```python
from build123d import *

# Parameters (mm, degrees)
SKETCH3_R           = 25
SKETCH3_R_2         = 72
BOSS_EXTRUDE1_DEPTH = 28
SKETCH4_R           = 10.5
CUT_EXTRUDE1_DEPTH  = 3671.216984417


with BuildPart() as part:
    # Sketch3 → Boss-Extrude1 (new body)
    with BuildSketch(Plane(origin=(0, 0, 0), x_dir=(1, 0, 0), z_dir=(0, 1, 0))):
        with BuildLine():
            Line((2845.680118699, 2169.501165066), (2845.680118699, 2074.501165066))
            ThreePointArc((2845.680118699, 2074.501165066), (2848.414414178, 2016.917733414), (2860.484776028, 1960.547223948))
            ThreePointArc((2860.484776028, 1960.547223948), (2949.180118699, 1699.501165066), (2860.484776028, 1438.455106185))
            ThreePointArc((2860.484776028, 1438.455106185), (2848.414414178, 1382.084596719), (2845.680118699, 1324.501165066))
            Line((2845.680118699, 1324.501165066), (2845.680118699, 1229.501165066))
            Line((2845.680118699, 1229.501165066), (2830.680118699, 1214.501165066))
            Line((2830.680118699, 1214.501165066), (2210.680118699, 1214.501165066))
            Line((2210.680118699, 1214.501165066), (2195.680118699, 1229.501165066))
            Line((2195.680118699, 1229.501165066), (2195.680118699, 1324.501165066))
            ThreePointArc((2195.680118699, 1324.501165066), (2192.94582322, 1382.084596719), (2180.87546137, 1438.455106185))
            ThreePointArc((2180.87546137, 1438.455106185), (2092.180118699, 1699.501165066), (2180.87546137, 1960.547223948))
            ThreePointArc((2180.87546137, 1960.547223948), (2192.94582322, 2016.917733414), (2195.680118699, 2074.501165066))
            Line((2195.680118699, 2074.501165066), (2195.680118699, 2169.501165066))
            Line((2195.680118699, 2169.501165066), (2210.680118699, 2184.501165066))
            Line((2210.680118699, 2184.501165066), (2830.680118699, 2184.501165066))
            Line((2830.680118699, 2184.501165066), (2845.680118699, 2169.501165066))
        make_face()
        with Locations(Location((2844.180118699, 1699.501165066, 0), (0, 0, 270))):
            Circle(SKETCH3_R, mode=Mode.SUBTRACT)
        with Locations(Location((2520.680118699, 1400.501165066, 0), (0, 0, 270))):
            Circle(SKETCH3_R_2, mode=Mode.SUBTRACT)
        with Locations(Location((2520.680118699, 1998.501165066, 0), (0, 0, 270))):
            Circle(SKETCH3_R_2, mode=Mode.SUBTRACT)
        with BuildLine():
            Line((2620.554891012, 1673.06787727), (2562.676931085, 1635.306037562))
            ThreePointArc((2562.676931085, 1635.306037562), (2520.680118699, 1622.914580714), (2478.683306313, 1635.306037562))
            Line((2478.683306313, 1635.306037562), (2420.805346386, 1673.06787727))
            ThreePointArc((2420.805346386, 1673.06787727), (2406.139786968, 1699.889370895), (2420.805346386, 1726.71086452))
            Line((2420.805346386, 1726.71086452), (2478.683306313, 1764.472704228))
            ThreePointArc((2478.683306313, 1764.472704228), (2520.680118699, 1776.864161076), (2562.676931085, 1764.472704228))
            Line((2562.676931085, 1764.472704228), (2620.554891012, 1726.71086452))
            ThreePointArc((2620.554891012, 1726.71086452), (2635.220450429, 1699.889370895), (2620.554891012, 1673.06787727))
        make_face(mode=Mode.SUBTRACT)
    extrude(amount=BOSS_EXTRUDE1_DEPTH)

    # Sketch4 → Cut-Extrude1 (cut, through all)
    with BuildSketch(Plane(origin=(0, 28, 0), x_dir=(1, 0, 0), z_dir=(0, 1, 0))):
        with Locations(Location((2520.680118699, 2099.501165066, 0), (0, 0, 270))):
            Circle(SKETCH4_R)
        with Locations(Location((2624.20773674, 2085.871495582, 0), (0, 0, 270))):
            Circle(SKETCH4_R)
        with Locations(Location((2720.680118699, 2045.91132658, 0), (0, 0, 270))):
            Circle(SKETCH4_R)
        with Locations(Location((2803.522831173, 1982.343877541, 0), (0, 0, 270))):
            Circle(SKETCH4_R)
        with Locations(Location((2867.090280213, 1899.501165066, 0), (0, 0, 270))):
            Circle(SKETCH4_R)
        with Locations(Location((2907.050449214, 1803.028783107, 0), (0, 0, 270))):
            Circle(SKETCH4_R)
        with Locations(Location((2920.680118699, 1699.501165066, 0), (0, 0, 270))):
            Circle(SKETCH4_R)
        with Locations(Location((2907.050449214, 1595.973547025, 0), (0, 0, 270))):
            Circle(SKETCH4_R)
        with Locations(Location((2867.090280213, 1499.501165066, 0), (0, 0, 270))):
            Circle(SKETCH4_R)
        with Locations(Location((2803.522831173, 1416.658452592, 0), (0, 0, 270))):
            Circle(SKETCH4_R)
        with Locations(Location((2720.680118699, 1353.091003552, 0), (0, 0, 270))):
            Circle(SKETCH4_R)
        with Locations(Location((2624.20773674, 1313.130834551, 0), (0, 0, 270))):
            Circle(SKETCH4_R)
        with Locations(Location((2520.680118699, 1299.501165066, 0), (0, 0, 270))):
            Circle(SKETCH4_R)
        with Locations(Location((2417.152500658, 1313.130834551, 0), (0, 0, 270))):
            Circle(SKETCH4_R)
        with Locations(Location((2320.680118699, 1353.091003552, 0), (0, 0, 270))):
            Circle(SKETCH4_R)
        with Locations(Location((2237.837406224, 1416.658452592, 0), (0, 0, 270))):
            Circle(SKETCH4_R)
        with Locations(Location((2174.269957185, 1499.501165066, 0), (0, 0, 270))):
            Circle(SKETCH4_R)
        with Locations(Location((2134.309788183, 1595.973547025, 0), (0, 0, 270))):
            Circle(SKETCH4_R)
        with Locations(Location((2120.680118699, 1699.501165066, 0), (0, 0, 270))):
            Circle(SKETCH4_R)
        with Locations(Location((2134.309788183, 1803.028783107, 0), (0, 0, 270))):
            Circle(SKETCH4_R)
        with Locations(Location((2174.269957185, 1899.501165066, 0), (0, 0, 270))):
            Circle(SKETCH4_R)
        with Locations(Location((2237.837406224, 1982.343877541, 0), (0, 0, 270))):
            Circle(SKETCH4_R)
        with Locations(Location((2320.680118699, 2045.91132658, 0), (0, 0, 270))):
            Circle(SKETCH4_R)
        with Locations(Location((2417.152500658, 2085.871495582, 0), (0, 0, 270))):
            Circle(SKETCH4_R)
    extrude(amount=-CUT_EXTRUDE1_DEPTH, mode=Mode.SUBTRACT)


solid = part.part
```
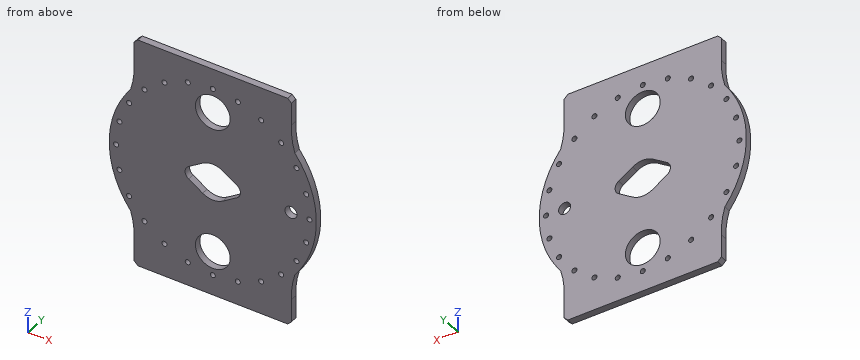
Geometry: final body of the model. Coordinates: model frame, mm. Coordinates: 2 decimals unless noted, no trailing zeros. Order: outer loops, then holes, each group sorted by start corner. A loop starts at its lowest first (then second) coordinate and runs counter-clockwise, first axis right, second up. Notation, with made-up numbers: M 60,14.25 L 87,14.25 A21 ccw 87,25.25 Z; hole C 68.5,55 d1. An arc over 180 degrees is marked long. Answer in a Markdown table with one row per item. Add a question column.
Q1. Section query A-A on z = -1596. Return the cut outline in (x, y), and give its area (3 significant figures).
Q2. Contact query for flat-ended pins moving along their axis: P1, Ø8, axis at y = 7.5, z = -2037, coming from the -X side; P2, Ø14, axis at y = 15.5, z = -1258, coming from the +X side; P3, Ø1, axis at y = 7, z = -1872, coming from the +X side. Output: stop coordinate, or through.
Q3. Section query B-B on y = 5. Count the separate pieces of the cut face and the enclosed holes in it, and give its area (3 significant figures).
Q4. Line query: L1, parallel to X at y = 27, z = -1989; L2, parallel to X at y = 14.5, z = -1422; L3, parallel to X at y = 23.25, z = -1490. Output: solid intervals per line, ascending.
Completed:
| question | item | result |
|---|---|---|
| 1 | outline | M 2104.87,0 L 2123.81,0 L 2123.81,28 L 2104.87,28 Z; M 2144.81,0 L 2896.55,0 L 2896.55,28 L 2144.81,28 Z; M 2917.55,0 L 2936.49,0 L 2936.49,28 L 2917.55,28 Z |
| 1 | area | 22,100 mm2 |
| 2 | P1 | stops at x = 2194.66 |
| 2 | P2 | stops at x = 2845.68 |
| 2 | P3 | stops at x = 2913.14 |
| 3 | separate pieces | 1 |
| 3 | enclosed holes | 28 |
| 3 | area | 644,000 mm2 |
| 4 | L1 | x = 2188.17 to 2229.72, 2245.96 to 2449.31, 2592.05 to 2795.4, 2811.64 to 2853.19 |
| 4 | L2 | x = 2185.4 to 2228.8, 2246.88 to 2451.96, 2589.4 to 2794.48, 2812.56 to 2855.96 |
| 4 | L3 | x = 2146.89 to 2169.8, 2178.74 to 2862.62, 2871.56 to 2894.47 |
